Read the model definition and answer for the solid it produces. Units are mm, in the model's axes. Face numbers are marked on the shaded views. Give positions to 0.01 mm unless a question says otherwise; leave off trailing zeros. Order: outer loops, then holes, each group sorted by start corner. A loop starts at its lowest first (then second) coordinate and runs counter-clockwise, first axis right, second up.
Item 1: A cutting plane is placed at B-B (x = 0). Write down the section's boundary in (y, z).
Item 2: The mould has two halves that part along Z. Classify the marked faces 1, 2 and 3: +Z half, -Z half, draft (parallel to the pull), parting line (faces both ways), or undercut.
Item 3: A cutting plane is placed at A-A (z = 24). Write down the section's boundary in (x, y), plus the area to 3 significant figures.
Item 4: Given pin 1 Ø15 at (x, z) = (0, -18.5) entering from -Y, flat-ended and moving along its own axis, determine where the tip first touches the part or whether it passes through.
Item 5: A cutting plane is placed at C-C (y = 2). State how many separate pieces and enclosed holes the cut face has, plus the area to 3 significant figures.
Item 6: Find the intervals of material crossed by line 1 along Z through (x, y) = (6, 4.25); line 2 along Z through (x, y) = (6.5, 2.25); line 3 along Z through (x, y) = (3.5, 0.5), in increasing order.
from build123d import *

# Parameters (mm, degrees)
SKETCH1_W                = 25
SKETCH1_H                = 75
BOSS_EXTRUDE1_DEPTH      = 8
SKETCH2_R                = 2.25
CUT_EXTRUDE1_DEPTH       = 20
SKETCH3_R                = 6.5
CUT_EXTRUDE2_DEPTH       = 20
SKETCH4_W                = 35.479601552
SKETCH4_H                = 10
CUT_EXTRUDE3_DEPTH       = 10
SKETCH5_W                = 25
SKETCH5_H                = 6.5
CUT_EXTRUDE4_DEPTH       = 10
CHAMFER1_SIZE            = 3
SKETCH6_R                = 1.6
CUT_EXTRUDE5_DEPTH       = 10
CIRPATTERN1_COUNT        = 4
SKETCH7_R                = 10.25
CUT_EXTRUDE6_DEPTH       = 3
SKETCH8_R                = 2.25
CUT_EXTRUDE7_DEPTH       = 36.72814017
CHAMFER2_SIZE            = 1
F_3_0_3_DIAMETER_HOLE1_D = 3
F_4_0_4_DIAMETER_HOLE1_D = 4
CUT_EXTRUDE8_DEPTH       = 36.72814017
CHAMFER3_SIZE            = 0.5
M3_TAPPED_HOLE1_D        = 2.5
M3_TAPPED_HOLE1_DEPTH    = 8.5
M3_TAPPED_HOLE1_TIP      = 0.751075774


with BuildPart() as part:
    # Sketch1 → Boss-Extrude1 (new body)
    with BuildSketch(Plane(origin=(0, 0, 0), x_dir=(1, 0, 0), z_dir=(0, 1, 0))):
        Rectangle(SKETCH1_W, SKETCH1_H)
    extrude(amount=BOSS_EXTRUDE1_DEPTH)

    # Sketch2 → Cut-Extrude1 (cut)
    with BuildSketch(Plane.XZ):
        with Locations(Location((-8, 24, 0), (0, 0, 270))):
            Circle(SKETCH2_R)
        with Locations(Location((8, 24, 0), (0, 0, 90))):
            Circle(SKETCH2_R)
    extrude(amount=-CUT_EXTRUDE1_DEPTH, mode=Mode.SUBTRACT)

    # Sketch3 → Cut-Extrude2 (cut)
    with BuildSketch(Plane(origin=(0, 8, 0), x_dir=(1, 0, 0), z_dir=(0, 1, 0))):
        with Locations(Location((0, 18.5, 0), (0, 0, 270))):
            Circle(SKETCH3_R)
    extrude(amount=-CUT_EXTRUDE2_DEPTH, mode=Mode.SUBTRACT)

    # Sketch4 → Cut-Extrude3 (cut)
    with BuildSketch(Plane(origin=(0, 8, 0), x_dir=(1, 0, 0), z_dir=(0, 1, 0))):
        with Locations((0, -37.5)):
            Rectangle(SKETCH4_W, SKETCH4_H)
    extrude(amount=-CUT_EXTRUDE3_DEPTH, mode=Mode.SUBTRACT)

    # Sketch5 → Cut-Extrude4 (cut)
    with BuildSketch(Plane(origin=(0, 8, 0), x_dir=(1, 0, 0), z_dir=(0, 1, 0))):
        with Locations((0, 34.25)):
            Rectangle(SKETCH5_W, SKETCH5_H)
    extrude(amount=-CUT_EXTRUDE4_DEPTH, mode=Mode.SUBTRACT)

    # Chamfer1
    chamfer1_edges = [part.edges().sort_by_distance(p)[0] for p in [
        (12.5, 4, 32.5),
        (-12.5, 4, 32.5),
    ]]
    chamfer(chamfer1_edges, length=CHAMFER1_SIZE)

    # Sketch6 → Cut-Extrude5 (cut)
    with BuildSketch(Plane.XZ):
        with Locations(Location((9.899494937, -8.600505063, 0), (0, 0, 270))):
            Circle(SKETCH6_R)
    cut_extrude5 = extrude(amount=-CUT_EXTRUDE5_DEPTH, mode=Mode.SUBTRACT)

    # CirPattern1: Cut-Extrude5 ×4 about axis
    cirpattern1_axis = Axis((0, 0, -18.5), (0, 1, 0))
    for i in range(1, CIRPATTERN1_COUNT):
        add(cut_extrude5.rotate(cirpattern1_axis, i * 360 / CIRPATTERN1_COUNT), mode=Mode.SUBTRACT)

    # Sketch7 → Cut-Extrude6 (cut)
    with BuildSketch(Plane.XZ):
        with Locations(Location((0, -18.5, 0), (0, 0, 270))):
            Circle(SKETCH7_R)
    extrude(amount=-CUT_EXTRUDE6_DEPTH, mode=Mode.SUBTRACT)

    # Sketch8 → Cut-Extrude7 (cut, through all)
    with BuildSketch(Plane(origin=(0, 8, 0), x_dir=(1, 0, 0), z_dir=(0, 1, 0))):
        with Locations(Location((-8, -1, 0), (0, 0, 270))):
            Circle(SKETCH8_R)
        with Locations(Location((8, -1, 0), (0, 0, 90))):
            Circle(SKETCH8_R)
    extrude(amount=-CUT_EXTRUDE7_DEPTH, mode=Mode.SUBTRACT)

    # Chamfer2
    chamfer2_edges = [part.edges().sort_by_distance(p)[0] for p in [
        (-12.5, 4, -31),
        (12.5, 4, -31),
    ]]
    chamfer(chamfer2_edges, length=CHAMFER2_SIZE)

    # Ø3.0 (3) Diameter Hole1 (through all)
    with Locations(Plane(origin=(0, 0, 0), x_dir=(-1, 0, 0), z_dir=(0, -1, 0))):
        with Locations((3, -1), (-3, -1)):
            Hole(F_3_0_3_DIAMETER_HOLE1_D / 2)

    # Ø4.0 (4) Diameter Hole1 (through all)
    with Locations(Plane(origin=(0, 0, 0), x_dir=(-1, 0, 0), z_dir=(0, -1, 0))):
        with Locations((0, -9)):
            Hole(F_4_0_4_DIAMETER_HOLE1_D / 2)

    # Sketch14 → Cut-Extrude8 (cut, through all)
    with BuildSketch(Plane(origin=(0, 8, 0), x_dir=(1, 0, 0), z_dir=(0, 1, 0))):
        with BuildLine():
            Line((2.75, 0.5), (3.25, 0.5))
            ThreePointArc((3.25, 0.5), (4.75, -1), (3.25, -2.5))
            Line((3.25, -2.5), (2.75, -2.5))
            ThreePointArc((2.75, -2.5), (1.25, -1), (2.75, 0.5))
        make_face()
    extrude(amount=-CUT_EXTRUDE8_DEPTH, mode=Mode.SUBTRACT)

    # Chamfer3
    chamfer3_edges = [part.edges().sort_by_distance(p)[0] for p in [
        (0, 0, -8.25),
        (0, 8, -25),
    ]]
    chamfer(chamfer3_edges, length=CHAMFER3_SIZE)

    # M3 Tapped Hole1
    with Locations(Plane(origin=(0, 8, 0), x_dir=(1, 0, 0), z_dir=(0, 1, 0))):
        with Locations((-9.1, 18.5), (9.1, 18.5)):
            Hole(M3_TAPPED_HOLE1_D / 2, depth=M3_TAPPED_HOLE1_DEPTH)
            with Locations((0, 0, -(M3_TAPPED_HOLE1_DEPTH + M3_TAPPED_HOLE1_TIP / 2))):  # 118° drill point
                Cone(0, M3_TAPPED_HOLE1_D / 2, M3_TAPPED_HOLE1_TIP, mode=Mode.SUBTRACT)


solid = part.part
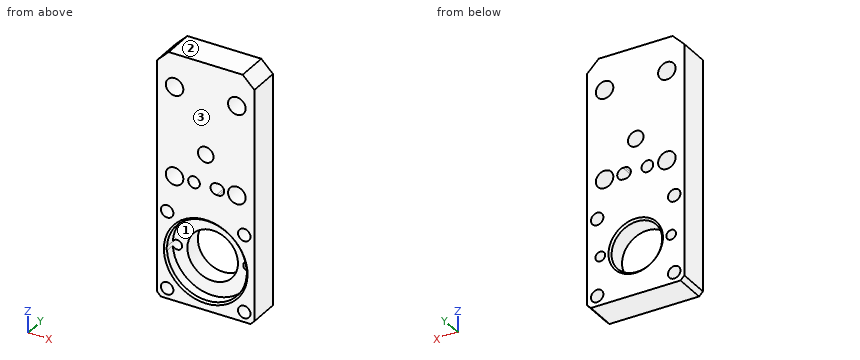
Response values:
1. outline: (0, -31) - (8, -31) - (8, -25.5) - (7.5, -25) - (3, -25) - (3, -28.75) - (0.5, -28.75) - (0, -29.25) - close; (0, -7.75) - (0.5, -8.25) - (3, -8.25) - (3, -12) - (7.5, -12) - (8, -11.5) - (8, 7) - (0, 7) - close; (0, 11) - (8, 11) - (8, 32.5) - (0, 32.5) - close
2. face 1: undercut
2. face 2: +Z half
2. face 3: draft
3. outline: (-12.5, 0) - (-10.25, 0) - (-10.25, 8) - (-12.5, 8) - close; (-5.75, 0) - (5.75, 0) - (5.75, 8) - (-5.75, 8) - close; (10.25, 0) - (12.5, 0) - (12.5, 8) - (10.25, 8) - close
3. area: 128 mm2
4. pin 1: stops at y = 3
5. separate pieces: 1
5. enclosed holes: 12
5. area: 1,120 mm2
6. line 1: z = -31 to -21, -16 to -0.03, 2.03 to 22.97, 25.03 to 32.5
6. line 2: z = -31 to -26.43, -10.57 to -0.68, 2.68 to 22.32, 25.68 to 32.5
6. line 3: z = -31 to -28.13, -8.87 to -0.48, 2.48 to 32.5
